Can you work these out from the model? Positions are in its coordinate system, mm. A direction names the side the tool comes from. Give positions to 0.01 mm unless a question says otherwise; leave off trailing zeros. Write each loop counter-clockwise with the first axis right and the second up, starting at its lowest first coordinate (ties: lowest second). Pieces come first, ordered by that corner, then holes.
```python
from build123d import *

# Parameters (mm, degrees)
SKETCH1_W               = 40
SKETCH1_H               = 80
BOSS_EXTRUDE1_DEPTH     = 45
SKETCH2_R               = 19
BOSS_EXTRUDE2_DEPTH     = 200
CUT_EXTRUDE1_DEPTH      = 248.436860633
CUT_EXTRUDE1_DEPTH_BACK = 248.436860633
SHELL1_T                = -2
SKETCH4_W               = 60
SKETCH4_H               = 100
SKETCH4_W_2             = 40
SKETCH4_H_2             = 80
BOSS_EXTRUDE3_DEPTH     = 2
CHAMFER1_SIZE           = 5
SKETCH5_R               = 1.75
CUT_EXTRUDE2_DEPTH      = 10
SKETCH6_R               = 1.75
CUT_EXTRUDE3_DEPTH      = 10
FILLET1_R               = 5


with BuildPart() as part:
    # Sketch1 → Boss-Extrude1 (new body)
    with BuildSketch(Plane.XY):
        Rectangle(SKETCH1_W, SKETCH1_H)
    extrude(amount=BOSS_EXTRUDE1_DEPTH)

    # Sketch2 → Boss-Extrude2 (add)
    with BuildSketch(Plane(origin=(0, 40, 0), x_dir=(1, 0, 0), z_dir=(0, 1, 0))):
        with Locations(Location((0, -25, 0), (0, 0, 90))):
            Circle(SKETCH2_R)
    extrude(amount=BOSS_EXTRUDE2_DEPTH)

    # Sketch3 → Cut-Extrude1 (cut, two sides: drawn at the far end of the back side and taken through both)
    with BuildSketch(Plane(origin=(20, 0, 0), x_dir=(0, 0, -1), z_dir=(1, 0, 0)).offset(-CUT_EXTRUDE1_DEPTH_BACK)):
        Polygon((200.08758149, -568.210195577), (-20, -40), (-45, 20), (-265.08758149, 548.210195577), (-1321.507972644, 108.035032596), (-856.332809663, -1008.385358557), align=None)
    extrude(amount=CUT_EXTRUDE1_DEPTH + CUT_EXTRUDE1_DEPTH_BACK, mode=Mode.SUBTRACT)

    # Shell1
    shell1_openings = [part.faces().sort_by_distance(p)[0] for p in [
        (0, 240, 25),
        (0, 0, 0),
    ]]
    offset(amount=SHELL1_T, openings=shell1_openings, kind=Kind.INTERSECTION)

    # Sketch4 → Boss-Extrude3 (add)
    with BuildSketch(Plane(origin=(0, 0, 0), x_dir=(-1, 0, 0), z_dir=(0, 0, -1))):
        Rectangle(SKETCH4_W, SKETCH4_H)
        Rectangle(SKETCH4_W_2, SKETCH4_H_2, mode=Mode.SUBTRACT)
    extrude(amount=-BOSS_EXTRUDE3_DEPTH)

    # Chamfer1
    chamfer1_edges = [part.edges().sort_by_distance(p)[0] for p in [
        (-30, -50, 1),
        (30, -50, 1),
        (30, 50, 1),
        (-30, 50, 1),
    ]]
    chamfer(chamfer1_edges, length=CHAMFER1_SIZE)

    # Sketch5 → Cut-Extrude2 (cut)
    with BuildSketch(Plane.XY.offset(2)):
        with Locations((-25, 0)):
            Circle(SKETCH5_R)
        with Locations((-25, 40)):
            Circle(SKETCH5_R)
        with Locations((-25, -40)):
            Circle(SKETCH5_R)
    cut_extrude2 = extrude(amount=-CUT_EXTRUDE2_DEPTH, mode=Mode.SUBTRACT)

    # Mirror1: Cut-Extrude2 across plane
    add(cut_extrude2.mirror(Plane(origin=(0, 0, 0), x_dir=(0, 0, 1), z_dir=(1, 0, 0))), mode=Mode.SUBTRACT)

    # Sketch6 → Cut-Extrude3 (cut)
    with BuildSketch(Plane.XY.offset(2)):
        with Locations((0, -45)):
            Circle(SKETCH6_R)
    extrude(amount=-CUT_EXTRUDE3_DEPTH, mode=Mode.SUBTRACT)

    # Sketch7 → Revolve1 (revolve)
    with BuildSketch(Plane(origin=(0, 0, 0), x_dir=(0, 0, -1), z_dir=(1, 0, 0))):
        Polygon((-44, 240), (-50.5, 290), (-50.5, 340), (-48.5, 340), (-48.5, 290.129455343), (-41.983170805, 240), align=None)
    revolve(axis=Axis((0, 340, 25), (0, -1, 0)))

    # Fillet1
    fillet1_edges = [part.edges().sort_by_distance(p)[0] for p in [
        (-20, 30, 45),
        (20, 30, 45),
        (20, -10, 32.5),
        (-20, -10, 32.5),
    ]]
    fillet(fillet1_edges, radius=FILLET1_R)


solid = part.part
```
1) For faces 1 (the face through (0, -40, 11)), 2 (the face through (13.127, 259.794, 7.88)), 3 (the face through (0, 29, 43)), 4 (the face through (-20, 8, 17)), which set-ups out of +Z, -Z, +X, -X, +Y, -Y let a thin tool reach every point of the face, with its end or its side?
Values follow:
face 1: +Z, +X, -X, -Y
face 2: none
face 3: -Z
face 4: +Z, -X, -Y
2) Please list where these lines run through material, in increasing order: L1, parallel to Y at x = -25, z = 1.25; L2, parallel to Z at x = 0, y = 321; L3, parallel to X at y = -18.5, z = 8.5.
Values follow:
L1: y = -50 to -41.75, -38.25 to -1.75, 1.75 to 38.25, 41.75 to 50
L2: z = -0.5 to 1.5, 48.5 to 50.5
L3: x = -20 to -18, 18 to 20
3) Suppose I cut it at A-A on y = 314. Write out the boundary of the cut face in (x, z), plus the area to 3 significant figures.
Values follow:
outline: circle Ø51 at (0, 25); hole circle Ø47 at (0, 25)
area: 308 mm2
4) For pin 1 Ø22 at (x, y) = (-4.5, 33.5) entering from +Z; pin 2 Ø4.5 at (x, y) = (-25, 40) entering from -Z; pin 3 Ø6 at (y, z) = (166.5, 37.5) entering from +X; pin 4 Ø3 at (x, y) = (25, 0) entering from -Z, each with a flat end and sliding along its axis, tell me the tip position at first contact or that it passes through.
Values follow:
pin 1: stops at z = 45
pin 2: stops at z = 0
pin 3: stops at x = 16.45
pin 4: passes through
5) If we mould it in two halves opening along X, with no side actions, what happens to faces 5 (the face through (20, 8, 17)), 6 (the face through (-0.21, -10.42, 32.325)), 7 (the face through (-0.888, 264.714, 4.824))? For each: +X half, -X half, draft (parallel to the pull), parting line (faces both ways), or undercut.
Values follow:
face 5: +X half
face 6: draft
face 7: undercut
